from build123d import *

# Parameters (mm, degrees)
SKETCH_1_R          = 3
EXTRUDE_1_DEPTH     = 12.75
CHAMFER_1_SIZE      = 0.2
SKETCH_2_R          = 2
EXTRUDE_2_DEPTH     = 7
CHAMFER_2_SIZE      = 0.2
SKETCH_3_R          = 5
EXTRUDE_3_DEPTH     = 8
CHAMFER_3_SIZE      = 0.2
CUT_EXTRUDE_1_REACH = 43.113
SKETCH_4_W          = 22.304994934
SKETCH_4_H          = 6.13630865
SKETCH_4_W_2        = 24.691337186
SKETCH_4_H_2        = 5.746701752
SKETCH_5_OUTSIDE_W  = 20.496
SKETCH_5_OUTSIDE_H  = 18.496
SKETCH_5_OUTSIDE_R  = 1.75
CUT_EXTRUDE_2_DEPTH = 1


with BuildPart() as part:
    # 草图1 → 凸台-拉伸1 (new, symmetric)
    with BuildSketch(Plane.XY):
        Circle(SKETCH_1_R)
    extrude(amount=EXTRUDE_1_DEPTH, both=True)

    # 倒角1
    chamfer_1_edges = [part.edges().sort_by_distance(p)[0] for p in [
        (-3, 0, -12.75),
    ]]
    chamfer(chamfer_1_edges, length=CHAMFER_1_SIZE)

    # 草图2 → 凸台-拉伸2 (add)
    with BuildSketch(Plane(origin=(0, 0, -12.75), x_dir=(-1, 0, 0), z_dir=(0, 0, -1))):
        with Locations(Location((0, 0, 0), (0, 0, 180))):
            Circle(SKETCH_2_R)
    extrude(amount=EXTRUDE_2_DEPTH)

    # 倒角2
    chamfer_2_edges = [part.edges().sort_by_distance(p)[0] for p in [
        (-2, 0, -19.75),
    ]]
    chamfer(chamfer_2_edges, length=CHAMFER_2_SIZE)

    # 草图3 → 凸台-拉伸3 (add)
    with BuildSketch(Plane.XY.offset(12.75)):
        Circle(SKETCH_3_R)
    extrude(amount=EXTRUDE_3_DEPTH)

    # 倒角3
    chamfer_3_edges = [part.edges().sort_by_distance(p)[0] for p in [
        (-5, 0, 12.75),
        (-5, 0, 20.75),
    ]]
    chamfer(chamfer_3_edges, length=CHAMFER_3_SIZE)

    # 切除-拉伸1: up to this face of the body (flat: up to its plane)
    cut_extrude_1_end = Plane(part.part.faces().sort_by_distance((-4.664235498, 0, 12.75))[0])
    # 草图4 → 切除-拉伸1 (cut, up to the picked face)
    with BuildSketch(Plane.XY.offset(20.75), mode=Mode.PRIVATE) as cut_extrude_1_sk1:
        with Locations((-4.583903449, 7.068154325)):
            Rectangle(SKETCH_4_W, SKETCH_4_H)
    cut_extrude_1_tool1 = split(extrude(cut_extrude_1_sk1.sketch, amount=-CUT_EXTRUDE_1_REACH, mode=Mode.PRIVATE), bisect_by=cut_extrude_1_end, keep=Keep.BOTH, mode=Mode.PRIVATE)
    # 草图4 → 切除-拉伸1 (cut, up to the picked face)
    with BuildSketch(Plane.XY.offset(20.75), mode=Mode.PRIVATE) as cut_extrude_1_sk2:
        with Locations((6.130286257, -6.873350876)):
            Rectangle(SKETCH_4_W_2, SKETCH_4_H_2)
    cut_extrude_1_tool2 = split(extrude(cut_extrude_1_sk2.sketch, amount=-CUT_EXTRUDE_1_REACH, mode=Mode.PRIVATE), bisect_by=cut_extrude_1_end, keep=Keep.BOTH, mode=Mode.PRIVATE)
    add(cut_extrude_1_tool1.solids().sort_by(Axis((-4.583903, 7.068154, 20.75), (0, 0, -1)))[0], mode=Mode.SUBTRACT)
    add(cut_extrude_1_tool2.solids().sort_by(Axis((6.130286, -6.873351, 20.75), (0, 0, -1)))[0], mode=Mode.SUBTRACT)

    # 草图5 outside → 切除-拉伸2 (cut)
    with BuildSketch(Plane(origin=(0, 0, -12.75), x_dir=(-1, 0, 0), z_dir=(0, 0, -1))):
        Rectangle(SKETCH_5_OUTSIDE_W, SKETCH_5_OUTSIDE_H)
        Circle(SKETCH_5_OUTSIDE_R, mode=Mode.SUBTRACT)
    extrude(amount=CUT_EXTRUDE_2_DEPTH, mode=Mode.SUBTRACT)


solid = part.part
The listing builds one solid part. Answer for the finished solid, in the listing's coordinates (mm). A direction names the side the tool comes from. Coordinates: 2 decimals unless noted, no trailing zeros. Write each loop counter-clockwise with the first axis right and the second up, starting at its lowest first coordinate (ties: lowest second). Pieces come first, ordered by that corner, then holes. Notation, with made-up numbers: M 55.5,89 L 106.5,89 A12 cw 106.5,103 Z; hole C 42.25,60.25 d4. An arc over 180 degrees is marked long. Put each result on its own line as item: value. Start each with the question number.
1. A cutting plane is placed at B-B on y = 0. Write down the section's boundary in (x, z).
2. A cutting plane is placed at D-D on z = -0.5. Write down the section's boundary in (x, y), then the cut area to 3 significant figures.
3. A cutting plane is placed at C-C on z = 17.5. Write down the section's boundary in (x, y), then the cut area to 3 significant figures.
4. For a pull along Z with two mould halves and no side action, classify faces 4 (the flat face through (0, 4, 17)), 5 (the flat face through (3, -1, 12.75)), 6 (the flat face through (0, -2, -12.75)) as pulls with the +Z half, pulls with the -Z half, needs draft (parallel to the pull), parting line crosses it, or undercut.
5. Which of the six approach directions +Z, -Z, +X, -X, +Y, -Y give full straight-line access (tool end or side, diameter ignored) to faces 1 (the cylindrical face through (5, 0, 17)), 2 (the cylindrical face through (-1.617, -0.67, -13.243)), 3 (the cylindrical face through (-3, 0, 0))?
6. A cutting plane is placed at A-A on x = 0. Write down the section's boundary in (y, z), then the cut area to 3 significant figures.
7. Consider line 1 (X direction, y = -3, z = 16); line 2 (Z direction, x = 2, y = -2.5); line 3 (Z direction, x = -1.75, y = 1.75). Determine where each line is inside the solid, lowest interval first. Write a range as from..to.
Resolved:
1. outline: M -5,12.95 L -4.8,12.75 L -3,12.75 L -3,-12.55 L -2.8,-12.75 L -1.75,-12.75 L -1.75,-13.75 L -2,-13.75 L -2,-19.55 L -1.8,-19.75 L 1.8,-19.75 L 2,-19.55 L 2,-13.75 L 1.75,-13.75 L 1.75,-12.75 L 2.8,-12.75 L 3,-12.55 L 3,12.75 L 4.8,12.75 L 5,12.95 L 5,20.55 L 4.8,20.75 L -4.8,20.75 L -5,20.55 Z
2. outline: C 0,0 d6
2. area: 28.3 mm2
3. outline: M -3,-4 L 3,-4 A5 ccw 3,4 L -3,4 A5 ccw Z
3. area: 70.4 mm2
4. face 4: needs draft
4. face 5: pulls with the -Z half
4. face 6: undercut
5. face 1: +Z, -Z, +X
5. face 2: none
5. face 3: -Z
6. outline: M -4,12.75 L -3,12.75 L -3,-12.55 L -2.8,-12.75 L -1.75,-12.75 L -1.75,-13.75 L -2,-13.75 L -2,-19.55 L -1.8,-19.75 L 1.8,-19.75 L 2,-19.55 L 2,-13.75 L 1.75,-13.75 L 1.75,-12.75 L 2.8,-12.75 L 3,-12.55 L 3,12.75 L 4,12.75 L 4,20.75 L -4,20.75 Z
6. area: 244 mm2
7. line 1: x = -4..4
7. line 2: z = 12.75..20.75
7. line 3: z = -12.75..20.75
